For this review, take the finished solid that the model builds, in its own axes (mm). Face numbers are marked on the shaded views. A direction names the side the tool comes from. Give positions to 0.01 mm unless a question says otherwise; leave off trailing zeros. Write each loop counter-clockwise with the first axis right and the second up, starting at its lowest first coordinate (ties: lowest second). Pieces come first, ordered by that corner, then holes.
Q1. We need section C-C (x = 67). Write out the cut boundary in (y, z).
Q2. Machinability: for the marked faces 3, 4 and 5, which of the approach directions +Z, -Z, +X, -X, +Y, -Y give a long, thin tool a straight path to every point of the face, cutting with its end or side? Answer none if there is none.
Q3. For line 1 (X direction, y = -0.5, z = 0.25); line 2 (Y direction, x = 77.5, z = -0.25); line 3 (X direction, y = 23, z = 3.5), list the stretches that pass through material, from the lowest coordinate up.
Q4. We need section A-A (y = 6). Write out the cut boundary in (x, z).
Q5. Insertion check: P1, Ø4, axis at x = -5.5, z = 1, coming from the -Y side; P2, Ø1.5, axis at x = 51, y = 29.5, coming from the -Z side; P3, Ø4, axis at x = 1.5, z = -2, coming from the +Y side. Each pin has a flat end and moves straight along its axis. Give the tip position at first contact, or say it passes through.
Q6. Mouldability with a two-part tool opening along X and no side actions: class the marked faces 1 and 2 as released by +X, released by -X, zero draft, split by the parting line, or undercut.
Q7. We need section B-B (z = 0). Write out the cut boundary in (x, y), then the cut area to 3 significant figures.
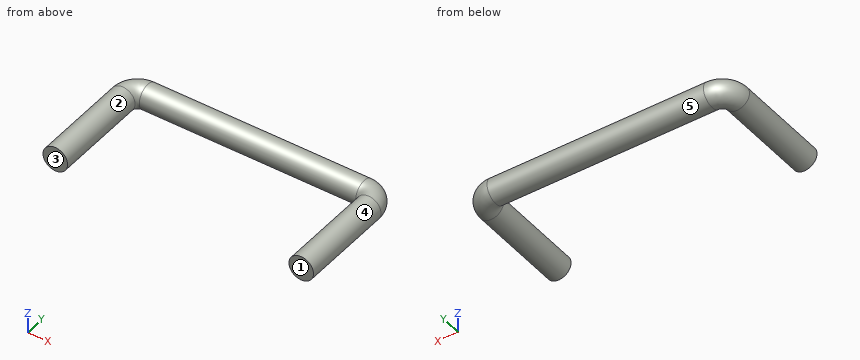
```python
from build123d import *

# Parameters (mm, degrees)
SKETCH2_R = 5


with BuildPart() as part:
    # Sweep1: sweep along a path in Sketch1
    with BuildLine(Plane.XY) as sweep1_path:
        Line((-15.997655985, -10.44225726), (-15.997655985, 28.55774274))
        ThreePointArc((-15.997655985, 28.55774274), (-14.240296673, 32.800383427), (-9.997655985, 34.55774274))
        Line((-9.997655985, 34.55774274), (78.002344015, 34.55774274))
        ThreePointArc((78.002344015, 34.55774274), (82.244984702, 32.800383427), (84.002344015, 28.55774274))
        Line((84.002344015, 28.55774274), (84.002344015, -10.44225726))
    # Sketch2 → Sweep1 (sweep)
    with BuildSketch(Plane(origin=(-15.997655985, -10.44225726, 0), x_dir=(-1, 0, 0), z_dir=(0, 1, 0))):
        Circle(SKETCH2_R)
    sweep(path=sweep1_path.line)


solid = part.part
```
Computed:
1. outline: circle Ø10 at (34.56, 0)
2. face 3: +Z, -Z, +X, -X, -Y
2. face 4: -Y
2. face 5: none
3. line 1: x = -20.99 to -11, 79.01 to 89
3. line 2: y = 29.56 to 39.55
3. line 3: x = -19.57 to -12.43, 80.43 to 87.57
4. outline: circle Ø10 at (-16, 0); circle Ø10 at (84, 0)
5. P1: stops at y = 29.56
5. P2: stops at z = -2.54
5. P3: stops at y = 39.56
6. face 1: zero draft
6. face 2: undercut
7. outline: (-21, -10.44) - (-11, -10.44) - (-11, 28.56) arc R1 cw to (-10, 29.56) - (78, 29.56) arc R1 cw to (79, 28.56) - (79, -10.44) - (89, -10.44) - (89, 28.56) arc R11 ccw to (78, 39.56) - (-10, 39.56) arc R11 ccw to (-21, 28.56) - close
7. area: 1,850 mm2
